```python
from build123d import *

# Parameters (mm, degrees)
SKETCH1_W             = 60
SKETCH1_H             = 124
BOSS_EXTRUDE1_DEPTH   = 5
SKETCH2_W             = 36
SKETCH2_H             = 102
CUT_EXTRUDE1_DEPTH    = 70.598850565
M4_TAPPED_HOLE1_D     = 3.3
M4_TAPPED_HOLE1_DEPTH = 10.1
M4_TAPPED_HOLE1_TIP   = 0.991420021
FILLET1_R             = 10
M4_TAPPED_HOLE2_D     = 3.3
M4_TAPPED_HOLE2_DEPTH = 10.1
M4_TAPPED_HOLE2_TIP   = 0.991420021
CHAMFER1_SIZE         = 1


with BuildPart() as part:
    # Sketch1 → Boss-Extrude1 (new, symmetric)
    with BuildSketch(Plane(origin=(0, 0, 0), x_dir=(0, 0, -1), z_dir=(1, 0, 0))):
        Rectangle(SKETCH1_W, SKETCH1_H)
    extrude(amount=BOSS_EXTRUDE1_DEPTH, both=True)

    # Sketch2 → Cut-Extrude1 (cut, through all)
    with BuildSketch(Plane(origin=(5, 0, 0), x_dir=(0, 0, -1), z_dir=(1, 0, 0))):
        Rectangle(SKETCH2_W, SKETCH2_H)
    extrude(amount=-CUT_EXTRUDE1_DEPTH, mode=Mode.SUBTRACT)

    # M4 Tapped Hole1
    with Locations(Plane(origin=(0, 62, 0), x_dir=(1, 0, 0), z_dir=(0, 1, 0))):
        with Locations((0, 0), (0, 21), (0, -21)):
            Hole(M4_TAPPED_HOLE1_D / 2, depth=M4_TAPPED_HOLE1_DEPTH)
            with Locations((0, 0, -(M4_TAPPED_HOLE1_DEPTH + M4_TAPPED_HOLE1_TIP / 2))):  # 118° drill point
                Cone(0, M4_TAPPED_HOLE1_D / 2, M4_TAPPED_HOLE1_TIP, mode=Mode.SUBTRACT)

    # Fillet1
    fillet1_edges = [part.edges().sort_by_distance(p)[0] for p in [
        (0, 51, -18),
        (0, -51, -18),
        (0, -51, 18),
        (0, 51, 18),
    ]]
    fillet(fillet1_edges, radius=FILLET1_R)

    # M4 Tapped Hole2
    with Locations(Plane(origin=(0, -62, 0), x_dir=(-1, 0, 0), z_dir=(0, -1, 0))):
        with Locations((0, 0), (0, 21), (0, -21)):
            Hole(M4_TAPPED_HOLE2_D / 2, depth=M4_TAPPED_HOLE2_DEPTH)
            with Locations((0, 0, -(M4_TAPPED_HOLE2_DEPTH + M4_TAPPED_HOLE2_TIP / 2))):  # 118° drill point
                Cone(0, M4_TAPPED_HOLE2_D / 2, M4_TAPPED_HOLE2_TIP, mode=Mode.SUBTRACT)

    # Chamfer1
    chamfer1_edges = [part.edges().sort_by_distance(p)[0] for p in [
        (0, -62, -30),
        (0, -62, 30),
        (0, 62, 30),
        (0, 62, -30),
    ]]
    chamfer(chamfer1_edges, length=CHAMFER1_SIZE)


solid = part.part
```
The listing builds one solid part. Answer for the finished solid, in the listing's coordinates (mm). A direction names the side the tool comes from. Give positions to 0.01 mm unless a question says otherwise; leave off trailing zeros. Loops run counter-clockwise (first coordinate to the right, second up) from the corner with the lowest first, then second, coordinate; pieces in that order, holes last. Notation, with made-up numbers: M 5,-2.75 L 33,-2.75 A16 ccw 33,12.25 Z; hole C -25.75,29.25 d6. An arc over 180 degrees is marked long. One line per item, written item: value.
1. For a pull along X with two mould halves and no side action, classify faces 4 (the face through (-0.04, 51.08, -21.28)), 5 (the face through (0, -1, 18)), 6 (the face through (0.215, 56.879, -22.636)), 7 (the face through (5, 1, 20)) as pulls with the +X half, pulls with the -X half, needs draft (parallel to the pull), parting line crosses it, or undercut.
Found:
face 4: undercut
face 5: needs draft
face 6: undercut
face 7: pulls with the +X half
2. Section B-B on z = -6 is taken. Determine the outline of the cut face in (x, y), plus the area to 3 significant figures.
Found:
outline: M -5,-62 L 5,-62 L 5,-51 L -5,-51 Z; M -5,51 L 5,51 L 5,62 L -5,62 Z
area: 220 mm^2
3. Each of these flat-tipped pins is pushed along its axis until it touches: P1, Ø4, axis at x = 0, z = -21, coming from the +Y side; P2, Ø2.5, axis at x = 0, z = -21, coming from the +Y side; P3, Ø2, axis at x = 0, z = 0, coming from the -Y side. Where does it stop, or does it pass through?
Found:
P1: y = 62
P2: y = 51.66
P3: y = -51.51
4. For faces 1 (the face through (-0.215, -56.879, -22.636)), 2 (the face through (0, -1, 30)), 3 (the face through (-0.07, 48.15, 14.99)), determine the directions among +Z, -Z, +X, -X, +Y, -Y from which every point of the face is accessible in a straight line to the end or side of a thin tool.
Found:
face 1: -Y
face 2: +Z, +X, -X, +Y, -Y
face 3: +X, -X
5. Section A-A on y = -17 is taken. Determine the outline of the cut face in (x, z), plus the area to 3 significant figures.
Found:
outline: M -5,-30 L 5,-30 L 5,-18 L -5,-18 Z; M -5,18 L 5,18 L 5,30 L -5,30 Z
area: 240 mm^2
6. Find the intervals of material crossed by probe 1 along Z at (x, y) = (0, -55); probe 2 along X at (y, z) = (-56.75, -21); probe 3 along Z at (x, y) = (1.5, -13.5), in increasing order.
Found:
probe 1: -30 to -22.65, -19.35 to -1.65, 1.65 to 19.35, 22.65 to 30
probe 2: -5 to -1.65, 1.65 to 5
probe 3: -30 to -18, 18 to 30
